```python
from build123d import *

# Parameters (mm, degrees)
SKETCH1_R           = 40
SKETCH1_R_2         = 30
BOSS_EXTRUDE1_DEPTH = 1.5
CHAMFER1_SIZE       = 0.3


with BuildPart() as part:
    # Sketch1 → Boss-Extrude1 (new, symmetric)
    with BuildSketch(Plane(origin=(0, 0, 0), x_dir=(1, 0, 0), z_dir=(0, 1, 0))):
        with Locations(Location((0, 0, 0), (0, 0, 270))):
            Circle(SKETCH1_R)
        with Locations(Location((0, 0, 0), (0, 0, 270))):
            Circle(SKETCH1_R_2, mode=Mode.SUBTRACT)
    extrude(amount=BOSS_EXTRUDE1_DEPTH, both=True)

    # Chamfer1
    chamfer1_edges = [part.edges().sort_by_distance(p)[0] for p in [
        (0, -1.5, -40),
        (0, 1.5, -40),
        (0, -1.5, -30),
        (0, 1.5, -30),
    ]]
    chamfer(chamfer1_edges, length=CHAMFER1_SIZE)


solid = part.part
```
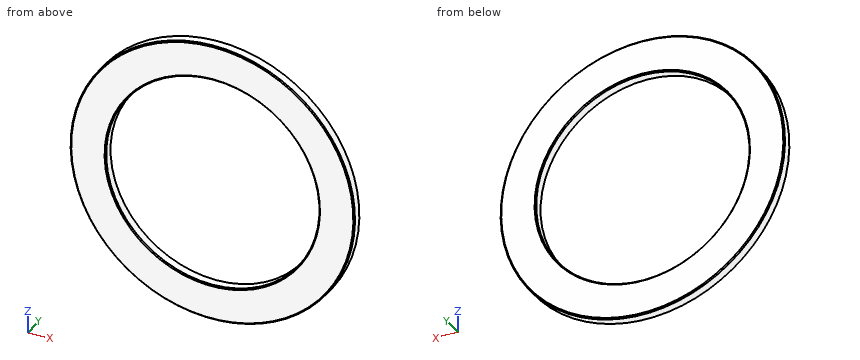
Part model, mm, in its own coordinate system. Round coordinates to 2 decimals unless told otherwise and drop trailing zeros. Loops run counter-clockwise (first coordinate to the right, second up) from the corner with the lowest first, then second, coordinate; pieces in that order, holes last.
Item 1: Drill centre lines: line 1 (X direction, y = 0.4, z = 0); line 2 (X direction, y = 0.35, z = 4.5); line 3 (Z direction, x = -6, y = -0.7). Where is each one in solid material? Low to high.
Item 2: Cut at B-B, the plane x = 0. Give the cut face in (y, z).
Item 3: Drop a flat-ended pin along its axis: P1, Ø1, axis at x = 16, y = 1, coming from the -Z side. Give the stop position or say it passes through.
Item 4: Cut at C-C, the plane y = 0.6. Give the cut face in (x, z), then the cut area to 3 significant figures.
Item 5: Cut at A-A, the plane z = 0. Give the cut face in (x, y), then the cut area to 3 significant figures.
A:
1. line 1: x = -40 to -30, 30 to 40
1. line 2: x = -39.75 to -29.66, 29.66 to 39.75
1. line 3: z = -39.55 to -29.39, 29.39 to 39.55
2. outline: (-1.5, -39.7) - (-1.2, -40) - (1.2, -40) - (1.5, -39.7) - (1.5, -30.3) - (1.2, -30) - (-1.2, -30) - (-1.5, -30.3) - close; (-1.5, 30.3) - (-1.2, 30) - (1.2, 30) - (1.5, 30.3) - (1.5, 39.7) - (1.2, 40) - (-1.2, 40) - (-1.5, 39.7) - close
3. P1: stops at z = -36.87
4. outline: circle Ø80 at (0, 0); hole circle Ø60 at (0, 0)
4. area: 2,200 mm2
5. outline: (-40, -1.2) - (-39.7, -1.5) - (-30.3, -1.5) - (-30, -1.2) - (-30, 1.2) - (-30.3, 1.5) - (-39.7, 1.5) - (-40, 1.2) - close; (30, -1.2) - (30.3, -1.5) - (39.7, -1.5) - (40, -1.2) - (40, 1.2) - (39.7, 1.5) - (30.3, 1.5) - (30, 1.2) - close
5. area: 59.6 mm2
